```python
from build123d import *

# Parameters (mm, degrees)
BOSS_EXTRUDE1_DEPTH                                 = 30
CBORE_FOR_M6_HEX_SOCKET_HEAD_CAP_SCREW1_D           = 6.6
CBORE_FOR_M6_HEX_SOCKET_HEAD_CAP_SCREW1_CBORE_D     = 11
CBORE_FOR_M6_HEX_SOCKET_HEAD_CAP_SCREW1_CBORE_DEPTH = 6.4
CHAMFER1_SIZE                                       = 2
CHAMFER2_SIZE                                       = 5


with BuildPart() as part:
    # Sketch1 → Boss-Extrude1 (new body)
    with BuildSketch(Plane.XY):
        Polygon((-25, 20), (-15, 20), (-15, 0), (15, 0), (15, 20), (25, 20), (25, -15), (-25, -15), align=None)
    extrude(amount=BOSS_EXTRUDE1_DEPTH)

    # CBORE for M6 Hex Socket Head Cap Screw1 (through all)
    with Locations(Plane.XY.offset(30)):
        with Locations((-15, -7), (15, -7)):
            CounterBoreHole(CBORE_FOR_M6_HEX_SOCKET_HEAD_CAP_SCREW1_D / 2, CBORE_FOR_M6_HEX_SOCKET_HEAD_CAP_SCREW1_CBORE_D / 2, CBORE_FOR_M6_HEX_SOCKET_HEAD_CAP_SCREW1_CBORE_DEPTH)

    # Chamfer1
    chamfer1_edges = [part.edges().sort_by_distance(p)[0] for p in [
        (-25, 20, 15),
        (-15, 20, 15),
        (15, 20, 15),
        (25, 20, 15),
    ]]
    chamfer(chamfer1_edges, length=CHAMFER1_SIZE)

    # Chamfer2
    chamfer2_edges = [part.edges().sort_by_distance(p)[0] for p in [
        (25, -15, 15),
        (-25, -15, 15),
    ]]
    chamfer(chamfer2_edges, length=CHAMFER2_SIZE)


solid = part.part
```
Geometry check sheet. Reference: the model listing, model coordinates, mm. A direction names the side the tool comes from. Give positions to 0.01 mm unless a question says otherwise; leave off trailing zeros. Order: outer loops, then holes, each group sorted by start corner. A loop starts at its lowest first (then second) coordinate and runs counter-clockwise, first axis right, second up.
1. Section check D-D, the plane x = -12.5. Enter the section's corners in (y, z), and give its area (3 significant figures).
2. Section check B-B, the plane z = 5.5. Enter the section's corners in (x, y), and give its area (3 significant figures).
3. Section check A-A, the plane y = -7. Enter the section's corners in (x, z).
4. Section check C-C, the plane y = 5. Enter the section's corners in (x, z).
5. Thickness scan on L1, parallel to X at y = 4, z = 3.75; L2, parallel to X at y = -11.5, z = 28; L3, parallel to X at y = -8, z = 28.25. Record the ranges inside material, lowest first.
6. Release check for a two-part mould opening along Y. For faces 4 (the face through (20.08, -9.11, 26.84)), 5 (the face through (23, -12, 15)), 6 (the face through (25, 4, 15)) record: pulls with the +Y half, pulls with the -Y half, needs draft (parallel to the pull), parting line crosses it, or undercut.
7. Gauge pin test, flat ends, axial feed: pin 1 Ø8 at (x, y) = (7, 6) entering from -Z; pin 2 Ø10 at (x, y) = (15, -7) entering from +Z; pin 3 Ø6 at (x, z) = (-13, 24) entering from +Y; pin 4 Ø1 at (x, z) = (8, 10) entering from +Y. Record the tip position at first contact, or that the pin passes through.
8. Access from +Z, -Z, +X, -X, +Y, -Y to the whole of each face (thin tool, end or side, straight path). Record for faces 1 (the face through (-16, 19, 15)), 2 (the face through (-25, 4, 15)), 3 (the face through (-16.19, -12.37, 26.84)).
Values follow:
1. outline: (-15, 0) - (-9.15, 0) - (-9.15, 23.6) - (-11.9, 23.6) - (-11.9, 30) - (-15, 30) - close; (-4.85, 0) - (0, 0) - (0, 30) - (-2.1, 30) - (-2.1, 23.6) - (-4.85, 23.6) - close
1. area: 286 mm2
2. outline: (-25, -10) - (-20, -15) - (20, -15) - (25, -10) - (25, 18) - (23, 20) - (17, 20) - (15, 18) - (15, 0) - (-15, 0) - (-15, 18) - (-17, 20) - (-23, 20) - (-25, 18) - close; hole circle Ø6.6 at (-15, -7); hole circle Ø6.6 at (15, -7)
2. area: 1,050 mm2
3. outline: (-25, 0) - (-18.3, 0) - (-18.3, 23.6) - (-20.5, 23.6) - (-20.5, 30) - (-25, 30) - close; (-11.7, 0) - (11.7, 0) - (11.7, 23.6) - (9.5, 23.6) - (9.5, 30) - (-9.5, 30) - (-9.5, 23.6) - (-11.7, 23.6) - close; (18.3, 0) - (25, 0) - (25, 30) - (20.5, 30) - (20.5, 23.6) - (18.3, 23.6) - close
4. outline: (-25, 0) - (-15, 0) - (-15, 30) - (-25, 30) - close; (15, 0) - (25, 0) - (25, 30) - (15, 30) - close
5. L1: x = -25 to -15, 15 to 25
5. L2: x = -23.5 to -18.16, -11.84 to 11.84, 18.16 to 23.5
5. L3: x = -25 to -20.41, -9.59 to 9.59, 20.41 to 25
6. face 4: undercut
6. face 5: pulls with the -Y half
6. face 6: needs draft
7. pin 1: passes through
7. pin 2: stops at z = 23.6
7. pin 3: stops at y = 19
7. pin 4: stops at y = 0
8. face 1: +Z, -Z, +Y
8. face 2: +Z, -Z, -X, +Y, -Y
8. face 3: +Z
